Input: dimensioned drawing with shaded views. Units: mm. Origin: part minimum x, y, z. A direction names the side the tool comes from. Round coordinates to 2 decimals unless told otherwise and drop trailing zeros. Loops run counter-clockwise (first coordinate to the right, second up) from the corner with the lowest first, then second, coordinate; pieces in that order, holes last. Notation, with made-up numbers: M -4.75,4.25 L 5.25,4.25 A10 ccw 5.25,21.25 Z; hole C -2,17.5 d1. An arc over 180 degrees is marked long. Answer as a JSON object with one key per item and string values.
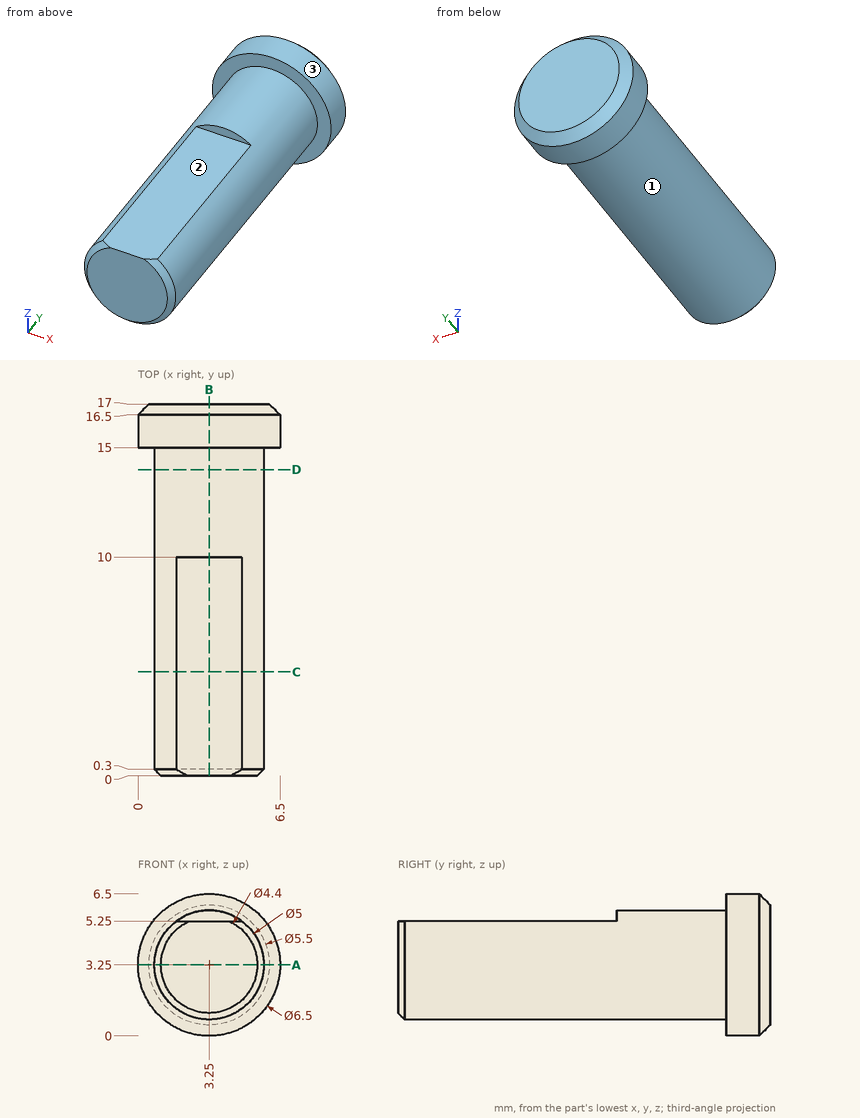
Item 1: Section C-C on y = 4.75. Return the cut outline in (x, z).
Answer sheet:
{"outline": "M 1.75,5.25 A2.5 ccw long 4.75,5.25 Z"}
Item 2: Section A-A on z = 3.25. Return the cut outline in (x, y), then the cut area to 3 significant figures.
Answer sheet:
{"outline": "M 0,15 L 0.75,15 L 0.75,0.3 L 1.05,0 L 5.45,0 L 5.75,0.3 L 5.75,15 L 6.5,15 L 6.5,16.5 L 6,17 L 0.5,17 L 0,16.5 Z", "area": "87.7 mm²"}
Item 3: Section B-B on x = 3.25. Return the cut outline in (y, z), then the cut area to 3 significant figures.
Answer sheet:
{"outline": "M 0,1.05 L 0.3,0.75 L 15,0.75 L 15,0 L 16.5,0 L 17,0.5 L 17,6 L 16.5,6.5 L 15,6.5 L 15,5.75 L 10,5.75 L 10,5.25 L 0,5.25 Z", "area": "82.7 mm²"}
Item 4: Access query for the marked faces 1, 2 and 3. Directions: +Z, -Z, +X, -X, +Y, -Y. A direction counts if a zero-diameter tool reaches every point of the face in a straight line with its end or side. Return the directions, or none.
Answer sheet:
{"face 1": "-Y", "face 2": "+Z, +X, -X, -Y", "face 3": "+Y, -Y"}
Item 5: Line query: probe 1 along Z at (x, y) = (1, 14.5); probe 2 along X at (y, z) = (6, 4); probe 3 along Z at (x, y) = (4.5, 1). Output: solid intervals per line, ascending. Write a range as from..to.
Answer sheet:
{"probe 1": "z = 2.16..4.34", "probe 2": "x = 0.87..5.63", "probe 3": "z = 1.08..5.25"}
Item 6: Contact query for flat-ended pins moving along their axis: pin 1 Ø2 at (x, y) = (1, 8) entering from -Z; pin 2 Ø2.5 at (x, y) = (3.5, 3) entering from +Z; pin 3 Ø2 at (y, z) = (12, 1.5) entering from +X. Output: stop coordinate, or through.
Answer sheet:
{"pin 1": "stops at z = 1.08", "pin 2": "stops at z = 5.25", "pin 3": "stops at x = 5.63"}
Item 7: Section D-D on y = 14. Return the cut outline in (x, z).
Answer sheet:
{"outline": "C 3.25,3.25 d5"}
